Could you check a few things on this model? Use its own coordinates, in mm. Face numbers are marked on the shaded views. A direction names the side the tool comes from. Give positions to 0.01 mm unless a question says otherwise; leave off trailing zeros. Order: outer loops, then holes, each group sorted by start corner. A loop starts at its lowest first (then second) coordinate and runs counter-clockwise, first axis right, second up. Notation, with made-up numbers: (50.5, 16) -> (101.5, 16) arc R25 cw to (101.5, 32) -> close; hole circle Ø6 at (47, 16). An arc over 180 degrees is marked (long way). Answer as CSV lines item,"result". Start each with the question number.
(1) I want a section at D-D (x = -6.5). Please give me the cut outline in (y, z).
(2) We'd pull the mould along X, two halves only. Please class the marked faces 3, 4 and 5: released by +X, released by -X, zero draft, split by the parting line, or undercut.
(3) I want a section at C-C (y = 1). Please give me the cut outline in (x, z).
(4) I want a section at B-B (x = 6.5). Please give me the cut outline in (y, z), plus the area to 3 significant figures.
(5) I need wall thicknesses on L1, parallel to Z at x = 6.5, y = 1; L2, parallel to Y at x = 1.25, z = 17; L3, parallel to Z at x = -4.5, y = 18. Which ranges of each line are inside material? Lowest first, please.
(6) I want a section at A-A (z = 9). Please give me the cut outline in (x, y), plus the area to 3 significant figures.
(7) Will these pins go through, and if not, where does the flat tip stop? pin 1 Ø8 at (x, z) = (6.5, 9) entering from +Y; pin 2 Ø10 at (y, z) = (28, 10.5) entering from +X; pin 3 Ø3 at (y, z) = (8, 14.5) entering from +X.
(8) On a 3-axis mill with a long thin cutter (end or side, diameter ignored), from which of +Z, -Z, +X, -X, +Y, -Y can I reach the whole of each face in a straight line? I mean the marked faces 1 and 2. Say none if no direction works.
```python
from build123d import *

# Parameters (mm, degrees)
SKETCH_1_W          = 25
SKETCH_1_H          = 10
EXTRUDE_1_DEPTH     = 18
SKETCH_2_R          = 4.5
EXTRUDE_2_DEPTH     = 30
CUT_EXTRUDE_1_REACH = 39.152
SKETCH_3_R          = 2.5
CHAMFER_1_SIZE      = 1


with BuildPart() as part:
    # 草图1 → 凸台-拉伸1 (new body)
    with BuildSketch(Plane.XY):
        Rectangle(SKETCH_1_W, SKETCH_1_H)
    extrude(amount=EXTRUDE_1_DEPTH)

    # 草图2 → 凸台-拉伸2 (add)
    with BuildSketch(Plane(origin=(0, 5, 0), x_dir=(1, 0, 0), z_dir=(0, 1, 0))):
        with Locations((-6.5, -9)):
            Circle(SKETCH_2_R)
    extrude(amount=EXTRUDE_2_DEPTH)

    # 草图3 → 切除-拉伸1 (cut, up to next)
    with BuildSketch(Plane(origin=(0, 5, 0), x_dir=(1, 0, 0), z_dir=(0, 1, 0)), mode=Mode.PRIVATE) as cut_extrude_1_sk1:
        with Locations(Location((6.5, -9, 0), (0, 0, 180))):
            Circle(SKETCH_3_R)
    cut_extrude_1_tool1 = extrude(cut_extrude_1_sk1.sketch, amount=-CUT_EXTRUDE_1_REACH, mode=Mode.PRIVATE) & part.part
    add(cut_extrude_1_tool1.solids().sort_by_distance((6.5, 5, 9))[0], mode=Mode.SUBTRACT)

    # 倒角1
    chamfer_1_edges = [part.edges().sort_by_distance(p)[0] for p in [
        (-12.5, 0, 18),
        (-12.5, 0, 0),
    ]]
    chamfer(chamfer_1_edges, length=CHAMFER_1_SIZE)


solid = part.part
```
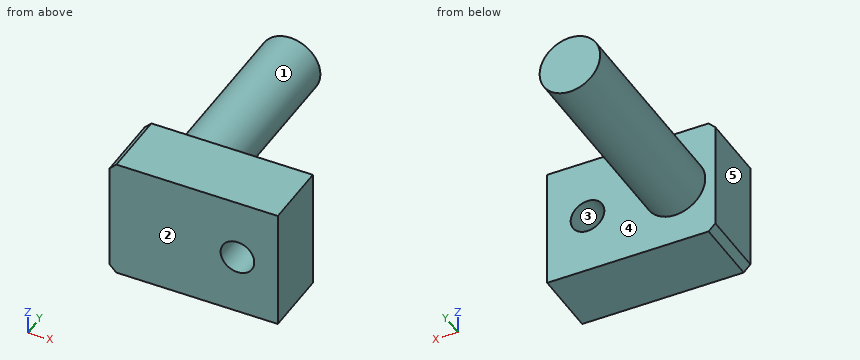
Final values:
1,outline,"(-5, 0) -> (5, 0) -> (5, 4.5) -> (35, 4.5) -> (35, 13.5) -> (5, 13.5) -> (5, 18) -> (-5, 18) -> close"
2,face 3,"undercut"
2,face 4,"zero draft"
2,face 5,"released by -X"
3,outline,"(-12.5, 1) -> (-11.5, 0) -> (12.5, 0) -> (12.5, 18) -> (-11.5, 18) -> (-12.5, 17) -> close; hole circle Ø5 at (6.5, 9)"
4,outline,"(-5, 0) -> (5, 0) -> (5, 6.5) -> (-5, 6.5) -> close; (-5, 11.5) -> (5, 11.5) -> (5, 18) -> (-5, 18) -> close"
4,area,"130 mm²"
5,L1,"0 to 6.5, 11.5 to 18"
5,L2,"-5 to 5"
5,L3,"4.97 to 13.03"
6,outline,"(-12.5, -5) -> (4, -5) -> (4, 5) -> (-2, 5) -> (-2, 35) -> (-11, 35) -> (-11, 5) -> (-12.5, 5) -> close; (9, -5) -> (12.5, -5) -> (12.5, 5) -> (9, 5) -> close"
6,area,"470 mm²"
7,pin 1,"y = 5"
7,pin 2,"x = -2"
7,pin 3,"x = -4.44"
8,face 1,"+Y"
8,face 2,"+Z, -Z, +X, -X, -Y"
